Verification items for the finished model (mm, model axes). Round coordinates to 2 decimals unless told otherwise and drop trailing zeros. Loops run counter-clockwise (first coordinate to the right, second up) from the corner with the lowest first, then second, coordinate; pieces in that order, holes last. Notation, with made-up numbers: M -11.75,85.25 L 29.25,85.25 A20 ccw 29.25,115.25 Z; hole C -6,82.5 d6. An arc over 180 degrees is marked long. One line per item, written item: value.
from build123d import *

# Parameters (mm, degrees)
SKETCH_1_W                = 690
SKETCH_1_H                = 1000
EXTRUDE_1_DEPTH           = 5
CHAMFER_1_SIZE            = 1
SKETCH_2_R                = 3
CUT_EXTRUDE_1_DEPTH       = 608.494855945
SKETCH_3_W                = 100
SKETCH_3_H                = 100
CUT_EXTRUDE_2_DEPTH       = 608.494855945
HOLE_WIZARD_6_0_6_1_D     = 6
HOLE_WIZARD_6_0_6_1_DEPTH = 5
HOLE_WIZARD_6_0_6_1_TIP   = 3
FILLET_1_R                = 10
SKETCH_6_W                = 30
SKETCH_6_H                = 500
CUT_EXTRUDE_3_DEPTH       = 10
CHAMFER_2_SIZE            = 1
FILLET_2_R                = 5


with BuildPart() as part:
    # 草图1 → 凸台-拉伸1 (new body)
    with BuildSketch(Plane(origin=(0, 0, 0), x_dir=(0, 0, -1), z_dir=(1, 0, 0))):
        Rectangle(SKETCH_1_W, SKETCH_1_H)
    extrude(amount=EXTRUDE_1_DEPTH)

    # 倒角1
    chamfer_1_edges = [part.edges().sort_by_distance(p)[0] for p in [
        (2.5, 500, 345),
        (2.5, 500, -345),
        (2.5, -500, -345),
        (2.5, -500, 345),
    ]]
    chamfer(chamfer_1_edges, length=CHAMFER_1_SIZE)

    # 草图2 → 切除-拉伸1 (cut, through all)
    with BuildSketch(Plane.ZY):
        with Locations(Location((-330, -485, 0), (0, 0, 180))):
            Circle(SKETCH_2_R)
        with Locations((330, -485)):
            Circle(SKETCH_2_R)
        with Locations(Location((330, 485, 0), (0, 0, 180))):
            Circle(SKETCH_2_R)
        with Locations((330, 0)):
            Circle(SKETCH_2_R)
        with Locations((-330, 0)):
            Circle(SKETCH_2_R)
    extrude(amount=-CUT_EXTRUDE_1_DEPTH, mode=Mode.SUBTRACT)

    # 草图3 → 切除-拉伸2 (cut, through all)
    with BuildSketch(Plane.ZY):
        with Locations((-295, -450)):
            Rectangle(SKETCH_3_W, SKETCH_3_H)
    extrude(amount=-CUT_EXTRUDE_2_DEPTH, mode=Mode.SUBTRACT)

    # Ø6.0 (6) 直径孔1
    with Locations(Plane(origin=(0, -600, 465), x_dir=(0, 0, 1), z_dir=(-1, 0, 0))):
        with Locations((-710, 1085), (-795, 1000), (-795, 300), (-610, 115)):
            Hole(HOLE_WIZARD_6_0_6_1_D / 2, depth=HOLE_WIZARD_6_0_6_1_DEPTH)
            with Locations((0, 0, -(HOLE_WIZARD_6_0_6_1_DEPTH + HOLE_WIZARD_6_0_6_1_TIP / 2))):  # 90° drill point
                Cone(0, HOLE_WIZARD_6_0_6_1_D / 2, HOLE_WIZARD_6_0_6_1_TIP, mode=Mode.SUBTRACT)

    # 圆角1
    fillet_1_edges = [part.edges().sort_by_distance(p)[0] for p in [
        (2.5, -400, -245),
    ]]
    fillet(fillet_1_edges, radius=FILLET_1_R)

    # 草图6 → 切除-拉伸3 (cut)
    with BuildSketch(Plane.ZY):
        with Locations((330, -250)):
            Rectangle(SKETCH_6_W, SKETCH_6_H)
    extrude(amount=-CUT_EXTRUDE_3_DEPTH, mode=Mode.SUBTRACT)

    # 倒角2
    chamfer_2_edges = [part.edges().sort_by_distance(p)[0] for p in [
        (2.5, -500, 315),
        (2.5, -500, -245),
        (2.5, -400, -345),
    ]]
    chamfer(chamfer_2_edges, length=CHAMFER_2_SIZE)

    # 圆角2
    fillet_2_edges = [part.edges().sort_by_distance(p)[0] for p in [
        (2.5, 0, 345),
        (2.5, 0, 315),
    ]]
    fillet(fillet_2_edges, radius=FILLET_2_R)


solid = part.part
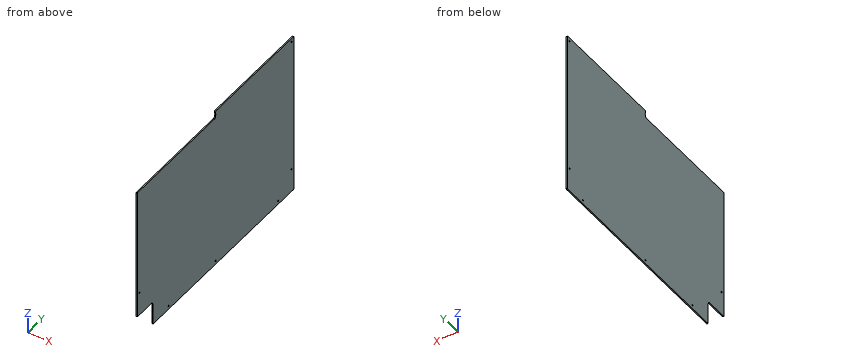
(1) Thickness scan on L1, parallel to Y at x = 2.3, z = -330; L2, parallel to Z at x = 4, y = 485; L3, parallel to Z at x = 2.9, y = -300. Record the ranges inside material, lowest first. Write a range as from..to.
Completed:
L1: y = -400..-303, -297..-3, 3..397, 403..500
L2: z = -345..-248, -242..327, 333..345
L3: z = -345..-333, -327..315
(2) Sectioned sample at B-B on y = -280.5. Enter the section's corners in (x, z), and give its area (3 significant figures).
Completed:
outline: M 0,-345 L 5,-345 L 5,315 L 0,315 Z
area: 3,300 mm^2
(3) Sectioned sample at A-A on x = 4.05. Enter the section's corners in (y, z).
Completed:
outline: M -500,-244 L -499,-245 L -410,-245 A10 cw -400,-255 L -400,-344 L -399,-345 L 499,-345 L 500,-344 L 500,344 L 499,345 L 5,345 A5 ccw 0,340 L 0,333 A3 cw 0,327 L 0,320 A5 cw -5,315 L -499,315 L -500,314 Z; hole C -485,-145 d6; hole C -300,-330 d6; hole C 0,-330 d6; hole C 400,-330 d6; hole C 485,-245 d6; hole C 485,330 d6
(4) Depth check by flat-ended pin: pin 1 Ø4 at (y, z) = (143.5, 67) entering from -X; pin 2 Ø1.5 at (x, z) = (3, 336) entering from -Y; pin 3 Ø1 at (x, y) = (1.5, -22.5) entering from +Z. Enter the tip coordinate at first touch or a pass-through.
Completed:
pin 1: stops at x = 0
pin 2: stops at y = 0
pin 3: stops at z = 315
